Check sheet for the modelled part. Datum: model origin and axes. Units: mm. Face numbers are marked on the shaded views. A direction names the side the tool comes from. Coordinates: 2 decimals unless noted, no trailing zeros. Loops run counter-clockwise (first coordinate to the right, second up) from the corner with the lowest first, then second, coordinate; pieces in that order, holes last.
```python
from build123d import *

# Parameters (mm, degrees)
CHAMFER_1_SIZE = 1
CHAMFER_2_SIZE = 0.5
CHAMFER_3_SIZE = 1


with BuildPart() as part:
    # 草图1 → 旋转1 (revolve)
    with BuildSketch(Plane(origin=(0, 0, 0), x_dir=(1, 0, 0), z_dir=(0, 1, 0)), mode=Mode.PRIVATE) as revolve_1_sk:
        Polygon((5.034928566, 40), (7.534928566, 40), (7.534928566, 42.5), (15.034928566, 42.5), (15.034928566, 37.5), (17.034928566, 37.5), (17.034928566, 38.5), (20.034928566, 38.5), (20.034928566, 37.5), (29.034928566, 37.5), (29.034928566, 42.5), (38.034928566, 42.5), (38.034928566, 37.5), (44.034928566, 37.5), (44.034928566, 46), (34.034928566, 46), (34.034928566, 47.5), (23.034928566, 47.5), (23.034928566, 46), (22.034928566, 46), (22.034928566, 51.5), (12.534928566, 51.5), (12.534928566, 51.75), (11.534928566, 51.75), (5.034928566, 48), align=None)
    revolve(revolve_1_sk.sketch.rotate(Axis((-85.103190975, 0, 0), (1, 0, 0)), 180), axis=Axis((-85.103190975, 0, 0), (1, 0, 0)))

    # 倒角1
    chamfer_1_edges = [part.edges().sort_by_distance(p)[0] for p in [
        (44.034928566, 0, -46),
    ]]
    chamfer(chamfer_1_edges, length=CHAMFER_1_SIZE)

    # 倒角2
    chamfer_2_edges = [part.edges().sort_by_distance(p)[0] for p in [
        (44.034928566, 0, -37.5),
    ]]
    chamfer(chamfer_2_edges, length=CHAMFER_2_SIZE)

    # 倒角3
    chamfer_3_edges = [part.edges().sort_by_distance(p)[0] for p in [
        (15.034928566, 0, -37.5),
    ]]
    chamfer(chamfer_3_edges, length=CHAMFER_3_SIZE)


solid = part.part
```
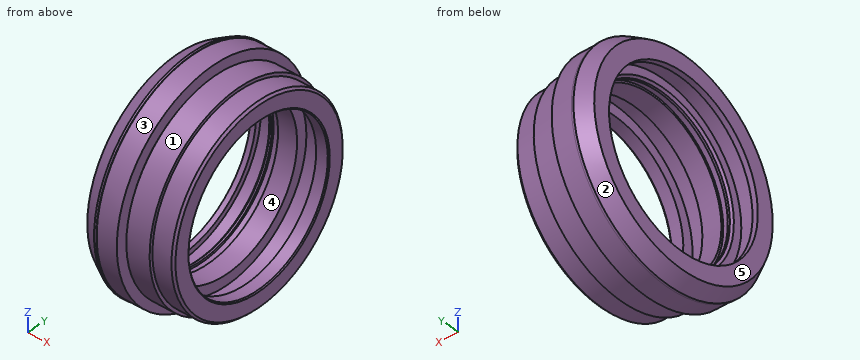
1) Scan lines: line 1 (X direction, y = -40, z = -10.5); line 2 (Y direction, x = 23.25, z = 0); line 3 (Y direction, x = 16, z = 0). Record each from-to range of solid material in increasing order.
Answer sheet:
line 1: x = 5.03 to 7.53, 15.03 to 29.03, 38.03 to 44.03
line 2: y = -47.5 to -37.5, 37.5 to 47.5
line 3: y = -51.5 to -37.53, 37.53 to 51.5
2) Set-up check for the marked faces 1 and 2: record each of +Z, -Z, +X, -X, +Y, -Y from which the full face is reachable in a straight line by a thin tool's end or side.
Answer sheet:
face 1: +X
face 2: -X
3) Mould release check, pull along Y, two halves, no side actions. Record for the marked faces 3, 4 and 5: +Y half, -Y half, draft (parallel to the pull), parting line (faces both ways), or undercut.
Answer sheet:
face 3: parting line
face 4: undercut
face 5: draft
4) Depth check by flat-ended pin: pin 1 (3 mm diameter, centred on x = 18, z = 34, fed in from -Y); pin 2 (1 mm diameter, centred on x = 20, y = -27.5, fed in from +Z); pin 3 (5 mm diameter, centred on x = 19.5, z = -27.5, fed in from -Y) (3 decimals). Enter the tip coordinate at first touch or a pass-through.
Answer sheet:
pin 1: stops at y = -39.95
pin 2: stops at z = 43.85
pin 3: stops at y = -45.025
5) Section check A-A on x = 24.5. Enter the section's corners in (y, z), plus the area to 3 significant figures.
Answer sheet:
outline: circle Ø95 at (0, 0); hole circle Ø75 at (0, 0)
area: 2,670 mm2
